Input: part model. Units: mm. Frame: model coordinates. Face numbers are marked on the shaded views. A direction names the side the tool comes from. Give positions to 0.01 mm unless a question says otherwise; leave off trailing zeros. Loops run counter-clockwise (first coordinate to the right, second up) from the corner with the lowest first, then second, coordinate; pieces in that order, holes last. Notation, with made-up numbers: M 37.5,11 L 91.5,11 A11 cw 91.5,31 Z; hole C 47.25,-29.5 d10. An arc over 180 degrees is marked long. Return JSON: item names as keys, results as strings. Group by question number.
```python
from build123d import *

# Parameters (mm, degrees)
SKETCH_2_R               = 6.25
CUT_EXTRUDE_1_DEPTH      = 122.548344291
PATTERN_CIRCULAR_1_COUNT = 4
CHAMFER_1_SIZE           = 1


with BuildPart() as part:
    # 草图1 → 旋转1 (revolve)
    with BuildSketch(Plane.XY, mode=Mode.PRIVATE) as revolve_1_sk:
        Polygon((0, 0), (0, 85), (13, 85), (13, 50), (18, 50), (18, 35), (13, 35), (13, 0), align=None)
    revolve(revolve_1_sk.sketch.rotate(Axis((0, 0, 0), (1, 0, 0)), 90), axis=Axis((0, 0, 0), (1, 0, 0)))

    # 草图2 → 切除-拉伸1 (cut, through all)
    with BuildSketch(Plane.ZY):
        with Locations((0, 70)):
            Circle(SKETCH_2_R)
    cut_extrude_1 = extrude(amount=-CUT_EXTRUDE_1_DEPTH, mode=Mode.SUBTRACT)

    # 阵列(圆周)1: 切除-拉伸1 ×4 about axis
    pattern_circular_1_axis = Axis((0, 0, 0), (1, 0, 0))
    for i in range(1, PATTERN_CIRCULAR_1_COUNT):
        add(cut_extrude_1.rotate(pattern_circular_1_axis, i * 360 / PATTERN_CIRCULAR_1_COUNT), mode=Mode.SUBTRACT)

    # 倒角1
    chamfer_1_edges = [part.edges().sort_by_distance(p)[0] for p in [
        (18, 0, -35),
        (18, 0, -50),
        (13, 0, -85),
        (0, 0, -85),
    ]]
    chamfer(chamfer_1_edges, length=CHAMFER_1_SIZE)


solid = part.part
```
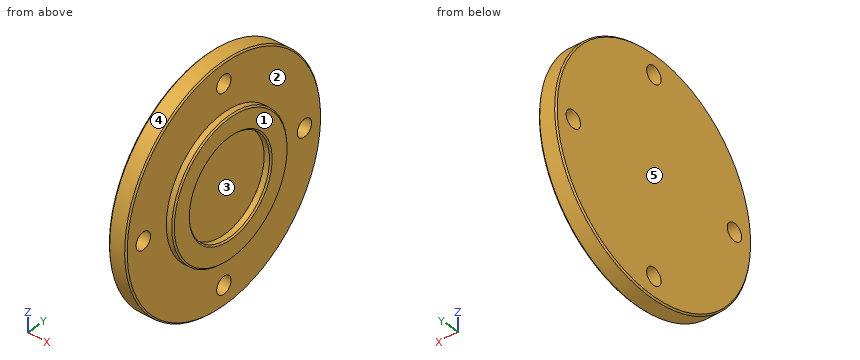
Item 1: Material intervals for line 1 (Y direction, x = 14.25, z = 0); line 2 (X direction, y = 55, z = 35.5); line 3 (Z direction, x = 10, y = -74), sorted ascending. Write a range as from..to.
Item 2: Section A-A, the plane z = 0. Return loops of the section in (x, y).
Item 3: Section C-C, the plane x = 5.5. Return loops of the section in (y, z).
Item 4: Pull-direction query (Y, two-part tool) for the marked faces 3, 4 and 5; classes: pulls with the +Y half, pulls with the -Y half, needs draft (parallel to the pull), parting line crosses it, or undercut.
Item 5: Reachability of the marked faces 1 and 2 from +Z, -Z, +X, -X, +Y, -Y: full face, straight path, thin tool, end or side. Return the list, or none.
Item 6: First-contact query: pin 1 Ø10 at (y, z) = (-70, 0) entering from +X; pin 2 Ø1.5 at (x, z) = (11.5, -26) entering from -Y; pin 3 Ø10 at (x, z) = (5, -66) entering from -Y; pin 4 Ø8 at (x, y) = (6.5, 22) entering from -Z. Flat tips, straight axial feed; report the tip coordinate or a pass-through.
Answer below:
{
 "1": {"line 1": "-50..-35, 35..50", "line 2": "0..13", "line 3": "-41.82..-4.8, 4.8..41.82"},
 "2": {"outline": "M 0,-84 L 1,-85 L 12,-85 L 13,-84 L 13,-76.25 L 0,-76.25 Z; M 0,-63.75 L 13,-63.75 L 13,-50 L 17,-50 L 18,-49 L 18,-36 L 17,-35 L 13,-35 L 13,35 L 17,35 L 18,36 L 18,49 L 17,50 L 13,50 L 13,63.75 L 0,63.75 Z; M 0,76.25 L 13,76.25 L 13,84 L 12,85 L 1,85 L 0,84 Z"},
 "3": {"outline": "C 0,0 d170; hole C -70,0 d12.5; hole C 0,-70 d12.5; hole C 0,70 d12.5; hole C 70,0 d12.5"},
 "4": {"face 3": "undercut", "face 4": "parting line crosses it", "face 5": "needs draft"},
 "5": {"face 1": "+Z, -Z, +X, +Y, -Y", "face 2": "+X"},
 "6": {"pin 1": "through", "pin 2": "y = -81.16", "pin 3": "y = -59.19", "pin 4": "z = -83.07"}
}
